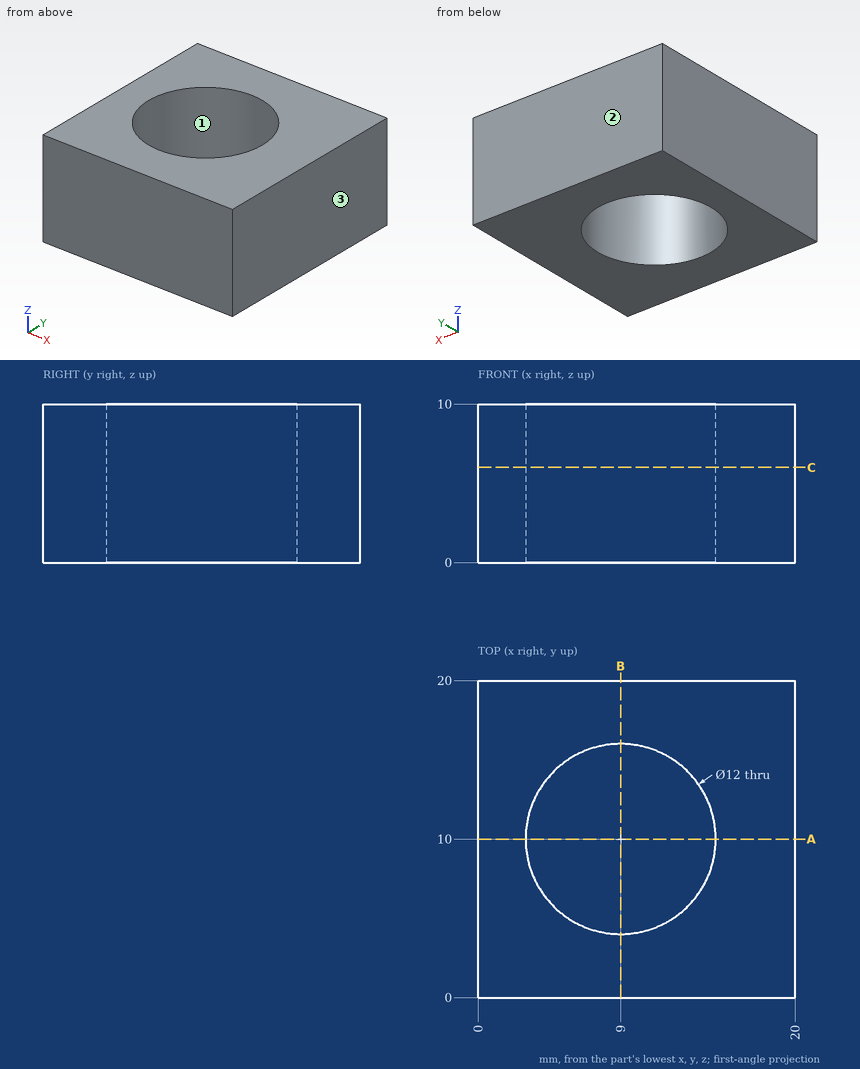
Here's the drawing with two shaded views (mm, measured from the low corner). I have some questions. Coordinates: 2 decimals unless noted, no trailing zeros. Order: outer loops, then holes, each group sorted by start corner. A loop starts at its lowest first (then second) coordinate and runs counter-clockwise, first axis right, second up. Notation, with made-up numbers: (-14.5, 79) - (24.5, 79) arc R23 cw to (24.5, 112) - close; hole circle Ø4 at (-37, 80.5). An arc over 180 degrees is marked (long way). Use CSV: the item, a comma, the result in double quotes. Start each with the question number.
1. Suppose I cut it at C-C on z = 6. List the corners of the cut face in (x, y) for me, then the cut area to 3 significant figures.
2. Suppose I cut it at A-A on y = 10. List the corners of the cut face in (x, z) for me.
3. Suppose I cut it at B-B on x = 9. List the corners of the cut face in (y, z) for me.
4. Please list where these lines run through material, in increasing order: line 1 (Y direction, x = 9, z = 6.75); line 2 (X direction, y = 12.25, z = 4); line 3 (Y direction, x = 11.75, z = 4.75). Write a range as from..to.
5. If we mould it in two halves opening along X, with no side actions, what happens to the marked faces 1, 2 and 3? For each: +X half, -X half, draft (parallel to the pull), parting line (faces both ways), or undercut.
Output:
1,outline,"(0, 0) - (20, 0) - (20, 20) - (0, 20) - close; hole circle Ø12 at (9, 10)"
1,area,"287 mm2"
2,outline,"(0, 0) - (3, 0) - (3, 10) - (0, 10) - close; (15, 0) - (20, 0) - (20, 10) - (15, 10) - close"
3,outline,"(0, 0) - (4, 0) - (4, 10) - (0, 10) - close; (16, 0) - (20, 0) - (20, 10) - (16, 10) - close"
4,line 1,"y = 0..4, 16..20"
4,line 2,"x = 0..3.44, 14.56..20"
4,line 3,"y = 0..4.67, 15.33..20"
5,face 1,"undercut"
5,face 2,"draft"
5,face 3,"+X half"
